Answer from the drawing. Dimensions are ordinates in mm from the lowest x, y and z of the part. Give positions to 0.01 mm unless a question says otherwise; leave off trailing zeros. Order: outer loops, then holes, each group sorted by start corner. A loop starts at its lowest first (then second) coordinate and runs counter-clockwise, first axis right, second up. Notation, with made-up numbers: (-17.5, 23) - (26.5, 23) arc R24 cw to (26.5, 42) - close; hole circle Ø6 at (74.5, -14.5). An arc over 180 degrees is marked (long way). Use a Markdown table: item, result. Add a question column.
1) Find section C-C, the plane z = 6. Determine the outline of the cut face in (x, y).
2) The mould has two halves that part along Y. Classify the marked faces 1, 2 and 3: released by +Y, released by -Y, zero draft, split by the parting line, or undercut.
3) Find section B-B, the plane y = 63. Determine the outline of the cut face in (x, z).
4) A flat-ended cylindrical pin translates along its axis: pin 1 (1 mm diameter, centred on y = 65, z = 7, fed in from -X). Find the tip coordinate at first contact, or state that the pin passes through.
5) Find section A-A, the plane z = 2.5. Determine the outline of the cut face in (x, y), plus the area to 3 significant figures.
6) Find section D-D, the plane x = 3. Determine the outline of the cut face in (y, z), plus the area to 3 significant figures.
7) Straight lines are drawn through the part: line 1 (Z direction, x = 48.5, y = 63); line 2 (Y direction, x = 50, z = 6); line 3 (Y direction, x = 27.5, z = 2.75). For each, find the intervals that lie inside material, in ascending order.
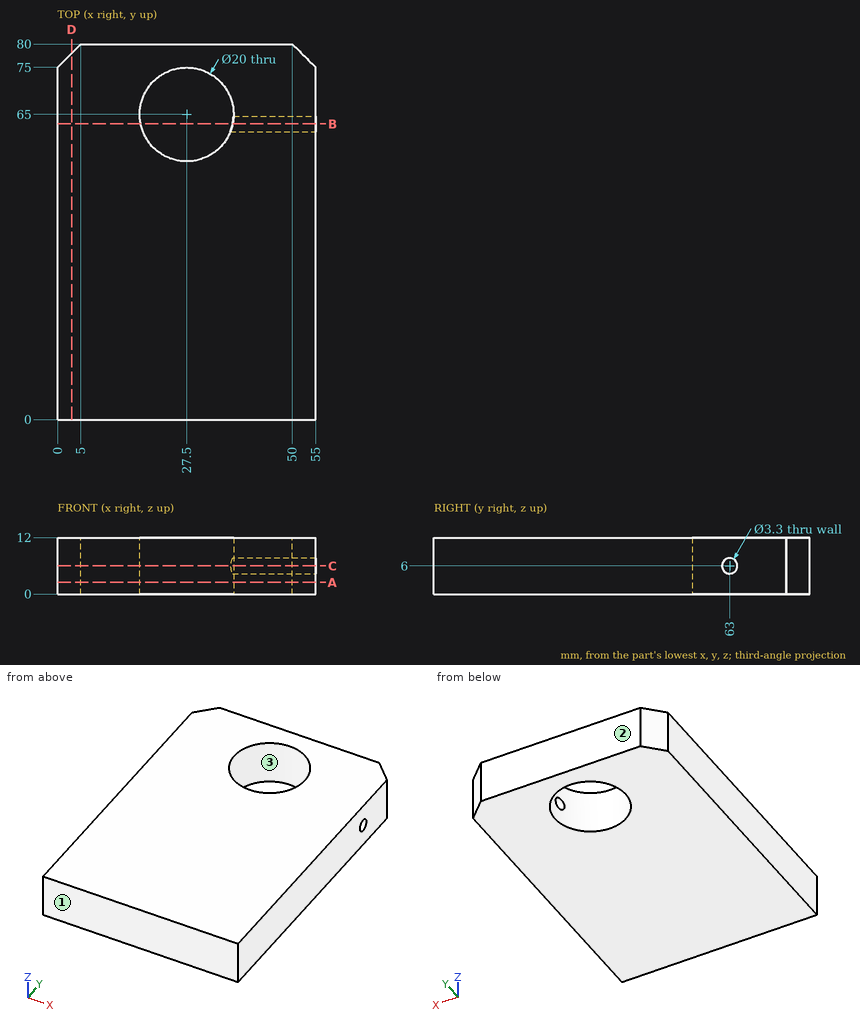
The answers:
| question | item | result |
|---|---|---|
| 1 | outline | (0, 0) - (55, 0) - (55, 61.35) - (36.81, 61.35) arc R10 cw (long way) to (37.49, 64.65) - (55, 64.65) - (55, 75) - (50, 80) - (5, 80) - (0, 75) - close |
| 2 | face 1 | released by -Y |
| 2 | face 2 | released by +Y |
| 2 | face 3 | undercut |
| 3 | outline | (0, 0) - (17.7, 0) - (17.7, 12) - (0, 12) - close; (37.3, 0) - (55, 0) - (55, 4.35) - (37.3, 4.35) - close; (37.3, 7.65) - (55, 7.65) - (55, 12) - (37.3, 12) - close |
| 4 | pin 1 | x = 0 |
| 5 | outline | (0, 0) - (55, 0) - (55, 75) - (50, 80) - (5, 80) - (0, 75) - close; hole circle Ø20 at (27.5, 65) |
| 5 | area | 4,060 mm2 |
| 6 | outline | (0, 0) - (78, 0) - (78, 12) - (0, 12) - close |
| 6 | area | 936 mm2 |
| 7 | line 1 | 0 to 4.35, 7.65 to 12 |
| 7 | line 2 | 0 to 61.35, 64.65 to 80 |
| 7 | line 3 | 0 to 55, 75 to 80 |
